Geometry: final body of the model. Coordinates: model frame, mm. Face numbers are marked on the shaded views. A direction names the side the tool comes from. Round coordinates to 2 decimals unless told otherwise and drop trailing zeros. Write each loop counter-clockwise with the first axis right and the second up, starting at its lowest first coordinate (ties: lowest second). Pieces come first, ordered by that corner, then holes. Notation, with made-up numbers: (81.25, 27) - (134.25, 27) arc R25 cw to (134.25, 45) - close; hole circle Ø4 at (65, 15.5). An arc over 180 degrees is marked (long way). Use a Markdown table: item, result. Add a question column.
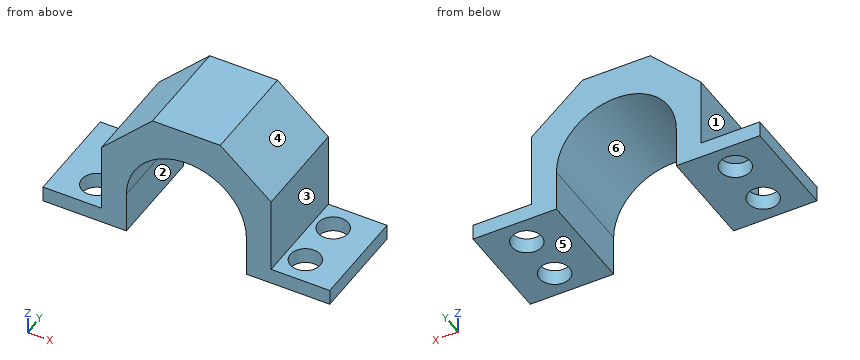
```python
from build123d import *

# Parameters (mm, degrees)
SADDLE_BODY_DEPTH       = 19.5
FLANGE_HOLES_SKETCH_R   = 5.754759715
FLANGE_BOLT_HOLES_DEPTH = 39


with BuildPart() as part:
    # Saddle Profile Sketch → Saddle Body (new, symmetric)
    with BuildSketch(Plane(origin=(0, 0, 0), x_dir=(1, 0, 0), z_dir=(0, 1, 0))):
        with BuildLine():
            Line((-23, -0.309929889), (-23, -16.309929889))
            ThreePointArc((-23, -16.309929889), (0, -39.309929889), (23, -16.309929889))
            Line((23, -16.309929889), (23, -0.309929889))
            Line((23, -0.309929889), (55, -0.309929889))
            Line((55, -0.309929889), (55, -6.309929889))
            Line((55, -6.309929889), (32.5, -6.309929889))
            Line((32.5, -6.309929889), (32.5, -35.619251923))
            Line((32.5, -35.619251923), (13, -52.309929889))
            Line((13, -52.309929889), (-13, -52.309929889))
            Line((-13, -52.309929889), (-32.5, -32.809929889))
            Line((-32.5, -32.809929889), (-32.5, -6.309929889))
            Line((-32.5, -6.309929889), (-55, -6.309929889))
            Line((-55, -6.309929889), (-55, -0.309929889))
            Line((-55, -0.309929889), (-23, -0.309929889))
        make_face()
    extrude(amount=SADDLE_BODY_DEPTH, both=True)

    # Flange Holes Sketch → Flange Bolt Holes (cut)
    with BuildSketch(Plane(origin=(0, 0, 0.309929889), x_dir=(-1, 0, 0), z_dir=(0, 0, -1))):
        with Locations((-40, 9.5)):
            Circle(FLANGE_HOLES_SKETCH_R)
        with Locations((40, 9.5)):
            Circle(FLANGE_HOLES_SKETCH_R)
        with Locations((40, -9.5)):
            Circle(FLANGE_HOLES_SKETCH_R)
        with Locations((-40, -9.5)):
            Circle(FLANGE_HOLES_SKETCH_R)
    extrude(amount=-FLANGE_BOLT_HOLES_DEPTH, mode=Mode.SUBTRACT)


solid = part.part
```
1) Set-up query: the marked faces 1, 2 and 3. Return all of +Z, -Z, +X, -X, +Y, -Y with unobstructed straight access to the full face (end or side cutting, diameter ignored); none if empty.
2) Section B-B, the plane x = 40. Return the cut outline in (y, z).
3) Section D-D, the plane z = 15. Return the cut outline in (x, y).
4) Section C-C, the plane z = 29.5. Return the cut outline in (x, y), then the cut area to 3 significant figures.
5) Draft query along X for the marked faces 4, 5 and 6. Return one class per face: released by +X, released by -X, zero draft, split by the parting line, or undercut.
6) Section A-A, the plane y = 9.5. Return the cut outline in (x, z).
7) Material intervals for L1, parallel to Y at x = 40, z = 3; L2, parallel to X at y = 9, z = 3; L3, parallel to X at y = -3, z = 11, sorted ascending. Write a range as from..to.
8) Pin query (flat end, axial travel): P1, Ø1.5, axis at y = 6, z = 42.5, coming from the +X side; P2, Ø21, axis at y = 9.5, z = 21, coming from the -X side; P3, Ø8, axis at y = -3.5, z = 8, coming from the +X side; P4, Ø14.5, axis at y = -1, z = 23, coming from the +X side. Return the tip coordinate at first contact, or that it passes through.
Output values:
| question | item | result |
|---|---|---|
| 1 | face 1 | +Z, -X, +Y, -Y |
| 1 | face 2 | -Z, +Y, -Y |
| 1 | face 3 | +Z, +X, +Y, -Y |
| 2 | outline | (-19.5, 0.31) - (-15.25, 0.31) - (-15.25, 6.31) - (-19.5, 6.31) - close; (-3.75, 0.31) - (3.75, 0.31) - (3.75, 6.31) - (-3.75, 6.31) - close; (15.25, 0.31) - (19.5, 0.31) - (19.5, 6.31) - (15.25, 6.31) - close |
| 3 | outline | (-32.5, -19.5) - (-23, -19.5) - (-23, 19.5) - (-32.5, 19.5) - close; (23, -19.5) - (32.5, -19.5) - (32.5, 19.5) - (23, 19.5) - close |
| 4 | outline | (-32.5, -19.5) - (-18.84, -19.5) - (-18.84, 19.5) - (-32.5, 19.5) - close; (18.84, -19.5) - (32.5, -19.5) - (32.5, 19.5) - (18.84, 19.5) - close |
| 4 | area | 1,070 mm^2 |
| 5 | face 4 | released by +X |
| 5 | face 5 | zero draft |
| 5 | face 6 | undercut |
| 6 | outline | (-55, 0.31) - (-45.75, 0.31) - (-45.75, 6.31) - (-55, 6.31) - close; (-34.25, 0.31) - (-23, 0.31) - (-23, 16.31) arc R23 cw to (23, 16.31) - (23, 0.31) - (34.25, 0.31) - (34.25, 6.31) - (32.5, 6.31) - (32.5, 35.62) - (13, 52.31) - (-13, 52.31) - (-32.5, 32.81) - (-32.5, 6.31) - (-34.25, 6.31) - close; (45.75, 0.31) - (55, 0.31) - (55, 6.31) - (45.75, 6.31) - close |
| 7 | L1 | y = -19.5..-15.25, -3.75..3.75, 15.25..19.5 |
| 7 | L2 | x = -55..-45.73, -34.27..-23, 23..34.27, 45.73..55 |
| 7 | L3 | x = -32.5..-23, 23..32.5 |
| 8 | P1 | stops at x = 25.34 |
| 8 | P2 | stops at x = -32.5 |
| 8 | P3 | stops at x = 55 |
| 8 | P4 | stops at x = 32.5 |
